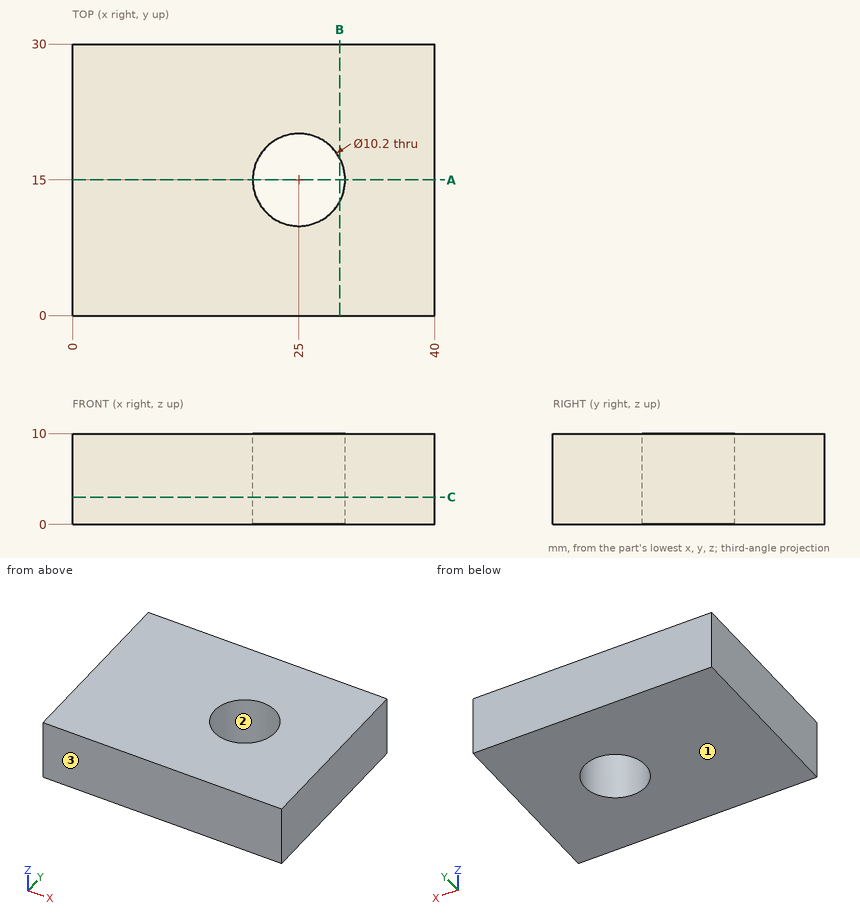
Answer from the drawing. Dimensions are ordinates in mm from the lowest x, y and z of the part. Round coordinates to 2 decimals unless told otherwise and drop trailing zeros. Order: outer loops, then holes, each group sorted by start corner. A loop starts at its lowest first (then second) coordinate and runs counter-clockwise, first axis right, second up. Notation, with made-up numbers: (45.25, -39) -> (99.25, -39) arc R17 cw to (99.25, -30) -> close; hole circle Ø8 at (-39.5, -24). An arc over 180 degrees is marked (long way). Answer as CSV lines item,"result".
Q1. A cutting plane is placed at C-C on z = 3. Determine the outline of the cut face in (x, y).
Computed values:
outline,"(0, 0) -> (40, 0) -> (40, 30) -> (0, 30) -> close; hole circle Ø10.2 at (25, 15)"
Q2. A cutting plane is placed at A-A on y = 15. Determine the outline of the cut face in (x, z), plus the area to 3 significant figures.
Computed values:
outline,"(0, 0) -> (19.9, 0) -> (19.9, 10) -> (0, 10) -> close; (30.1, 0) -> (40, 0) -> (40, 10) -> (30.1, 10) -> close"
area,"298 mm^2"
Q3. Consider line 1 (Y direction, x = 25, z = 6); line 2 (X direction, y = 13.75, z = 4.5); line 3 (Y direction, x = 27.5, z = 5.5). Determine where each line is inside the solid, lowest interval first. Write a range as from..to.
Computed values:
line 1,"y = 0..9.9, 20.1..30"
line 2,"x = 0..20.06, 29.94..40"
line 3,"y = 0..10.55, 19.45..30"
Q4. Given pin 1 (1 mm diameter, centred on x = 6.5, z = 6, fed in from -Y), flat-ended and moving along its own axis, determine where the tip first touches the part or whether it passes through.
Computed values:
pin 1,"stops at y = 0"
Q5. For a pull along Y with two mould halves and no side action, classify the marked faces 1, 2 and 3 as +Y half, -Y half, draft (parallel to the pull), parting line (faces both ways), or undercut.
Computed values:
face 1,"draft"
face 2,"undercut"
face 3,"-Y half"
Q6. A cutting plane is placed at B-B on x = 29.5. Determine the outline of the cut face in (y, z), plus the area to 3 significant figures.
Computed values:
outline,"(0, 0) -> (12.6, 0) -> (12.6, 10) -> (0, 10) -> close; (17.4, 0) -> (30, 0) -> (30, 10) -> (17.4, 10) -> close"
area,"252 mm^2"
